For this review, take the finished solid that the model builds, in its own axes (mm). A direction names the side the tool comes from. Coordinates: 2 decimals unless noted, no trailing zeros. Loops run counter-clockwise (first coordinate to the right, second up) from the corner with the lowest first, then second, coordinate; pieces in that order, holes last.
1. Take a section at A-A, the plane z = 0. State the section outline as (x, y) points.
2. To check wall thickness, follow probe 1 along Y at (x, z) = (0, -19); probe 2 along X at (y, z) = (1.55, 0); probe 3 along X at (y, z) = (20, 20). State the ranges of each line that lie inside material, in increasing order.
3. Take a section at C-C, the plane y = 18. State the section outline as (x, z) points, then the cut area to 3 significant figures.
4. Clearance check with flat-ended pins moving along their axes: P1, Ø1.5, axis at y = 25.5, z = 2.5, coming from the +X side; P2, Ø8, axis at y = 26, z = 15, coming from the -X side; P3, Ø12, axis at x = -21.5, y = 5, coming from the -Z side. State where each tip first meets the part, or that it passes through.
5. Machinability: for faces 1 (the face through (5.2, 30, 14.4)), 2 (the face through (-7.509, 2.465, 23.846)), 3 (the face through (25, 10, -7)), which of the approach directions +Z, -Z, +X, -X, +Y, -Y give a long, thin tool a straight path to every point of the face, cutting with its end or side? Answer none if there is none.
6. Mouldability with a two-part tool opening along X and no side actions: class faces 4 (the face through (7.509, 18.381, 23.846)), 5 (the face through (-5, 20, -19)), 6 (the face through (25, 0, -7)), 7 (the face through (-0.651, 24.957, 19.647)) as pulls with the +X half, pulls with the -X half, needs draft (parallel to the pull), parting line crosses it, or undercut.
7. Take a section at B-B, the plane x = 0. State the section outline as (y, z) points, then the cut area to 3 significant figures.
8. Take a section at D-D, the plane y = 9. State the section outline as (x, z) points.
```python
from build123d import *

# Parameters (mm, degrees)
FLANGE_PROFILE_60_R      = 30
BASE_FLANGE_60X10_DEPTH  = 10
BOSS_PROFILE_50_R        = 25
COLLAR_BOSS_50X20_DEPTH  = 20
BOSS_EDGE_FILLET_R3_R    = 3
CROSS_HOLE_PROFILE_10_R  = 5
CROSS_HOLE_10_DEPTH      = 35
COUNTERBORE_PROFILE_50_R = 25
COUNTERBORE_50X5_DEPTH   = 5
BORE_PROFILE_30_R        = 15
THROUGH_BORE_30_DEPTH    = 94


with BuildPart() as part:
    # Flange Profile Ø60 → Base Flange Ø60x10 (new body)
    with BuildSketch(Plane(origin=(0, 0, 0), x_dir=(1, 0, 0), z_dir=(0, 1, 0))):
        with Locations(Location((0, 0, 0), (0, 0, 270))):
            Circle(FLANGE_PROFILE_60_R)
    extrude(amount=BASE_FLANGE_60X10_DEPTH)

    # Boss Profile Ø50 → Collar Boss Ø50x20 (add)
    with BuildSketch(Plane(origin=(0, 10, 0), x_dir=(1, 0, 0), z_dir=(0, 1, 0))):
        with Locations(Location((0, 0, 0), (0, 0, 270))):
            Circle(BOSS_PROFILE_50_R)
    extrude(amount=COLLAR_BOSS_50X20_DEPTH)

    # Boss Edge Fillet R3
    boss_edge_fillet_r3_edges = [part.edges().sort_by_distance(p)[0] for p in [
        (0, 30, -25),
    ]]
    fillet(boss_edge_fillet_r3_edges, radius=BOSS_EDGE_FILLET_R3_R)

    # Cross Hole Profile Ø10 → Cross Hole Ø10 (cut, symmetric)
    with BuildSketch(Plane.XY):
        with Locations((0, 20)):
            Circle(CROSS_HOLE_PROFILE_10_R)
    extrude(amount=CROSS_HOLE_10_DEPTH, both=True, mode=Mode.SUBTRACT)

    # Counterbore Profile Ø50 → Counterbore Ø50x5 (cut)
    with BuildSketch(Plane.XZ):
        with Locations(Location((0, 0, 0), (0, 0, 90))):
            Circle(COUNTERBORE_PROFILE_50_R)
    extrude(amount=-COUNTERBORE_50X5_DEPTH, mode=Mode.SUBTRACT)

    # Bore Profile Ø30 → Through Bore Ø30 (cut)
    with BuildSketch(Plane.XZ.offset(-5)):
        with Locations(Location((0, 0, 0), (0, 0, 270))):
            Circle(BORE_PROFILE_30_R)
    extrude(amount=-THROUGH_BORE_30_DEPTH, mode=Mode.SUBTRACT)


solid = part.part
```
Results list:
1. outline: (-30, 0) - (-25, 0) - (-25, 5) - (-15, 5) - (-15, 30) - (-22, 30) arc R3 ccw to (-25, 27) - (-25, 10) - (-30, 10) - close; (15, 5) - (25, 5) - (25, 0) - (30, 0) - (30, 10) - (25, 10) - (25, 27) arc R3 ccw to (22, 30) - (15, 30) - close
2. probe 1: y = 5 to 15, 25 to 30
2. probe 2: x = -30 to -25, 25 to 30
2. probe 3: x = -15 to -5, 5 to 15
3. outline: (-4.58, -24.58) - (-4.58, -14.28) arc R15 cw to (-4.58, 14.28) - (-4.58, 24.58) arc R25 ccw to start; (4.58, -24.58) arc R25 ccw to (4.58, 24.58) - (4.58, 14.28) arc R15 cw to (4.58, -14.28) - close
3. area: 1,070 mm2
4. P1: stops at x = 24.94
4. P2: stops at x = -22.45
4. P3: stops at z = -25.69
5. face 1: +Z, -Z, +X, -X, +Y
5. face 2: -Y
5. face 3: +Y
6. face 4: parting line crosses it
6. face 5: undercut
6. face 6: needs draft
6. face 7: undercut
7. outline: (0, -30) - (10, -30) - (10, -25) - (15, -25) - (15, -15) - (5, -15) - (5, -25) - (0, -25) - close; (0, 25) - (5, 25) - (5, 15) - (15, 15) - (15, 25) - (10, 25) - (10, 30) - (0, 30) - close; (25, -25) - (27, -25) arc R3 ccw to (30, -22) - (30, -15) - (25, -15) - close; (25, 15) - (30, 15) - (30, 22) arc R3 ccw to (27, 25) - (25, 25) - close
7. area: 396 mm2
8. outline: circle Ø60 at (0, 0); hole circle Ø30 at (0, 0)
